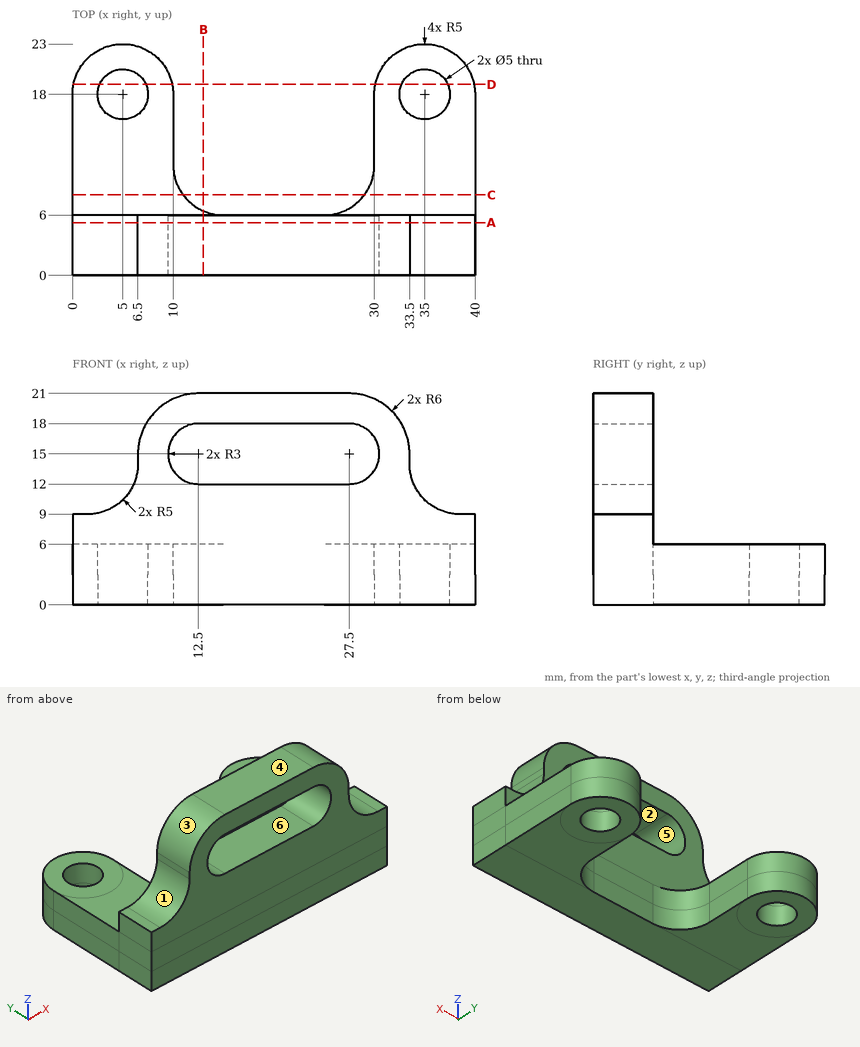
The drawing under review shows one solid part. Ordinate dimensions are in mm from its lowest x, y, z. A direction names the side the tool comes from. Round coordinates to 2 decimals unless told otherwise and drop trailing zeros. Loops run counter-clockwise (first coordinate to the right, second up) from the corner with the lowest first, then second, coordinate; pieces in that order, holes last.
Item 1: For line 1 (Y direction, x = 5, z = 1.5); line 2 (Z direction, x = 18, y = 1.5); line 3 (Y direction, x = 24.5, z = 8.25), list the stretches that pass through material, from the lowest coordinate up.
Determined:
line 1: y = 0 to 15.5, 20.5 to 23
line 2: z = 0 to 12, 18 to 21
line 3: y = 0 to 6
Item 2: Mouldability with a two-part tool opening along X and no side actions: class the marked faces 3, 4, 5 and 6 as released by +X, released by -X, zero draft, split by the parting line, or undercut.
Determined:
face 3: released by -X
face 4: zero draft
face 5: undercut
face 6: undercut
Item 3: Take a section at B-B (x = 13). Write out the cut boundary in (y, z), then the cut area to 3 significant figures.
Determined:
outline: (0, 0) - (6.42, 0) - (6.42, 6) - (6, 6) - (6, 12) - (0, 12) - close; (0, 18) - (6, 18) - (6, 21) - (0, 21) - close
area: 92.5 mm2
Item 4: Take a section at A-A (y = 5.25). Write out the cut boundary in (x, z), then the cut area to 3 significant figures.
Determined:
outline: (0, 0) - (40, 0) - (40, 9) - (38.5, 9) arc R5 cw to (33.5, 14) - (33.5, 15) arc R6 ccw to (27.5, 21) - (12.5, 21) arc R6 ccw to (6.5, 15) - (6.5, 14) arc R5 cw to (1.5, 9) - (0, 9) - close; hole (12.5, 12) - (27.5, 12) arc R3 ccw to (27.5, 18) - (12.5, 18) arc R3 ccw to start
area: 561 mm2
Item 5: Take a section at C-C (y = 8). Write out the cut boundary in (x, z).
Determined:
outline: (0, 0) - (11, 0) - (11, 6) - (0, 6) - close; (29, 0) - (40, 0) - (40, 6) - (29, 6) - close
Item 6: For the marked faces 1 and 2, list the 3-axis set-ups (+Z, -Z, +X, -X, +Y, -Y) from which the entire face can be reached by the end or side of a thin tool; tool diameter is ignored.
Determined:
face 1: +Z, -X, +Y, -Y
face 2: +Y, -Y
Item 7: Clearance check with flat-ended pins moving along their axes: pin 1 Ø6 at (x, z) = (16.5, 6) entering from +Y; pin 2 Ø12 at (x, z) = (10.5, 10.5) entering from +Y; pin 3 Ø3 at (x, z) = (20.5, 18) entering from +Y; pin 4 Ø4 at (y, z) = (9, 8.5) entering from +X (1 decimal). State where each tip first meets the part, or that it passes through.
Determined:
pin 1: stops at y = 6.23
pin 2: stops at y = 22.76
pin 3: stops at y = 6
pin 4: passes through
Item 8: Take a section at D-D (y = 19). Write out the cut boundary in (x, z).
Determined:
outline: (0.1, 0) - (2.71, 0) - (2.71, 6) - (0.1, 6) - close; (7.29, 0) - (9.9, 0) - (9.9, 6) - (7.29, 6) - close; (30.1, 0) - (32.71, 0) - (32.71, 6) - (30.1, 6) - close; (37.29, 0) - (39.9, 0) - (39.9, 6) - (37.29, 6) - close
